Input: part model. Units: mm. Frame: model coordinates. Face numbers are marked on the shaded views. A direction names the side the tool comes from. Coordinates: 2 decimals unless noted, no trailing zeros. Write each loop counter-clockwise with the first axis right and the second up, starting at its lowest first coordinate (ties: lowest second). Pieces come first, ordered by that corner, then holes.
1) Pin query (flat end, axial travel): pin 1 Ø3 at (y, z) = (4, 8.5) entering from -X; pin 2 Ø6 at (x, z) = (0, 26) entering from -Y; pin 3 Ø1 at (y, z) = (-6.5, 20) entering from +X; pin 4 Ø4 at (x, y) = (5, 2.5) entering from -Z. Return the tip coordinate at first contact, or that it passes through.
2) Section query A-A (y = 0). Output: boundary loops of the cut face in (x, z), then the cut area to 3 significant figures.
3) Section query C-C (z = 11). Output: boundary loops of the cut face in (x, y).
4) Set-up query: the marked faces 1 and 2. Return all of +Z, -Z, +X, -X, +Y, -Y with unobstructed straight access to the full face (end or side cutting, diameter ignored); none if empty.
5) Line query: L1, parallel to Z at x = -3.75, y = 8.5; L2, parallel to Y at x = 2.75, z = 26.5; L3, parallel to X at y = 6.5, z = 29. Output: solid intervals per line, ascending.
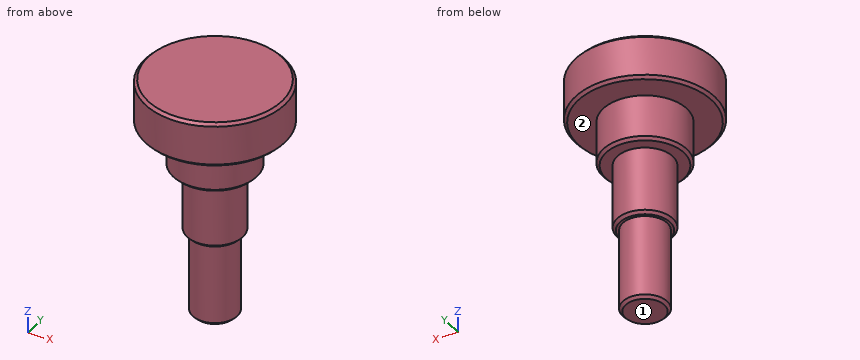
from build123d import *

# Parameters (mm, degrees)
SKETCH1_R           = 4
BOSS_EXTRUDE1_DEPTH = 15
SKETCH2_R           = 5
BOSS_EXTRUDE2_DEPTH = 12
SKETCH3_R           = 7.5
BOSS_EXTRUDE3_DEPTH = 8
SKETCH4_R           = 12.5
BOSS_EXTRUDE4_DEPTH = 8
CHAMFER1_SIZE       = 0.5


with BuildPart() as part:
    # Sketch1 → Boss-Extrude1 (new body)
    with BuildSketch(Plane.XY):
        Circle(SKETCH1_R)
    extrude(amount=BOSS_EXTRUDE1_DEPTH)

    # Sketch2 → Boss-Extrude2 (add)
    with BuildSketch(Plane.XY.offset(15)):
        Circle(SKETCH2_R)
    extrude(amount=BOSS_EXTRUDE2_DEPTH)

    # Sketch3 → Boss-Extrude3 (add)
    with BuildSketch(Plane.XY.offset(27)):
        Circle(SKETCH3_R)
    extrude(amount=BOSS_EXTRUDE3_DEPTH)

    # Sketch4 → Boss-Extrude4 (add)
    with BuildSketch(Plane.XY.offset(35)):
        Circle(SKETCH4_R)
    extrude(amount=BOSS_EXTRUDE4_DEPTH)

    # Chamfer1
    chamfer1_edges = [part.edges().sort_by_distance(p)[0] for p in [
        (-12.5, 0, 35),
        (-12.5, 0, 43),
        (-4, 0, 0),
        (-5, 0, 15),
        (-7.5, 0, 27),
    ]]
    chamfer(chamfer1_edges, length=CHAMFER1_SIZE)


solid = part.part
Answer:
1. pin 1: stops at x = -3.12
1. pin 2: stops at y = -7.5
1. pin 3: passes through
1. pin 4: stops at z = 0.09
2. outline: (-12.5, 35.5) - (-12, 35) - (-7.5, 35) - (-7.5, 27.5) - (-7, 27) - (-5, 27) - (-5, 15.5) - (-4.5, 15) - (-4, 15) - (-4, 0.5) - (-3.5, 0) - (3.5, 0) - (4, 0.5) - (4, 15) - (4.5, 15) - (5, 15.5) - (5, 27) - (7, 27) - (7.5, 27.5) - (7.5, 35) - (12, 35) - (12.5, 35.5) - (12.5, 42.5) - (12, 43) - (-12, 43) - (-12.5, 42.5) - close
2. area: 559 mm2
3. outline: circle Ø8 at (0, 0)
4. face 1: -Z, +X, -X, +Y, -Y
4. face 2: -Z
5. L1: z = 35 to 43
5. L2: y = -4.18 to 4.18
5. L3: x = -3.74 to 3.74
